```python
from build123d import *

# Parameters (mm, degrees)
SKETCH1_R           = 50
BOSS_EXTRUDE1_DEPTH = 5
SKETCH2_R           = 5
CUT_EXTRUDE1_DEPTH  = 5
CIRPATTERN1_COUNT   = 3
SKETCH3_R           = 9
CUT_EXTRUDE2_DEPTH  = 5


with BuildPart() as part:
    # Sketch1 → Boss-Extrude1 (new body)
    with BuildSketch(Plane.XY):
        Circle(SKETCH1_R)
    extrude(amount=BOSS_EXTRUDE1_DEPTH)

    # Sketch2 → Cut-Extrude1 (cut)
    with BuildSketch(Plane.XY.offset(5)):
        with Locations((0, 35)):
            Circle(SKETCH2_R)
    cut_extrude1 = extrude(amount=-CUT_EXTRUDE1_DEPTH, mode=Mode.SUBTRACT)

    # CirPattern1: Cut-Extrude1 ×3 about axis
    cirpattern1_axis = Axis((0, 0, 0), (0, 0, 1))
    for i in range(1, CIRPATTERN1_COUNT):
        add(cut_extrude1.rotate(cirpattern1_axis, i * 360 / CIRPATTERN1_COUNT), mode=Mode.SUBTRACT)

    # Sketch3 → Cut-Extrude2 (cut)
    with BuildSketch(Plane.XY.offset(5)):
        Circle(SKETCH3_R)
    extrude(amount=-CUT_EXTRUDE2_DEPTH, mode=Mode.SUBTRACT)


solid = part.part
```
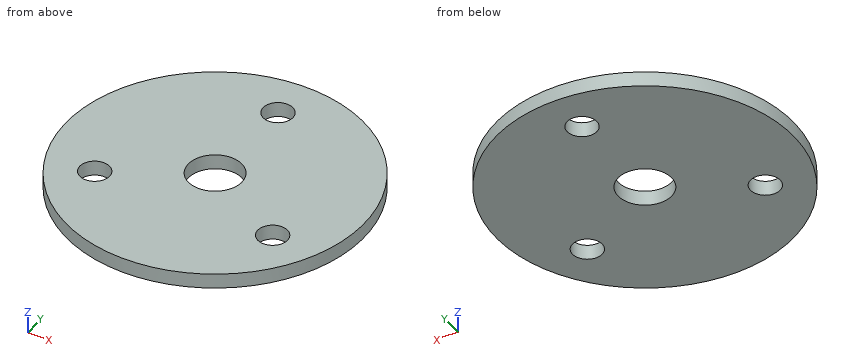
Input: part model. Units: mm. Frame: model coordinates. Give positions to 0.01 mm unless a question says otherwise; leave off trailing zeros. Order: outer loops, then holes, each group sorted by start corner. A loop starts at its lowest first (then second) coordinate and runs counter-clockwise, first axis right, second up.
1. Cut plane A-A (y = 0). Return loops of the section in (x, z).
Computed:
outline: (-50, 0) - (-9, 0) - (-9, 5) - (-50, 5) - close; (9, 0) - (50, 0) - (50, 5) - (9, 5) - close
2. Cut plane B-B (x = 0). Return loops of the section in (y, z), and give its area (3 significant figures).
Computed:
outline: (-50, 0) - (-9, 0) - (-9, 5) - (-50, 5) - close; (9, 0) - (30, 0) - (30, 5) - (9, 5) - close; (40, 0) - (50, 0) - (50, 5) - (40, 5) - close
area: 360 mm2
3. Line query: probe 1 along Y at (x, z) = (0, 3.25); probe 2 along X at (y, z) = (-0.5, 1.55); probe 3 along Y at (x, z) = (3, 0.4). Output: solid intervals per line, ascending.
Computed:
probe 1: y = -50 to -9, 9 to 30, 40 to 50
probe 2: x = -50 to -8.99, 8.99 to 50
probe 3: y = -49.91 to -8.49, 8.49 to 31, 39 to 49.91
4. Cut plane D-D (y = 35). Return loops of the section in (x, z), and give its area (3 significant figures).
Computed:
outline: (-35.71, 0) - (-5, 0) - (-5, 5) - (-35.71, 5) - close; (5, 0) - (35.71, 0) - (35.71, 5) - (5, 5) - close
area: 307 mm2
5. Pin query (flat end, axial travel): pin 1 Ø3 at (x, z) = (-17.5, 3) entering from -Y. Return the tip coordinate at first contact, or that it passes through.
Computed:
pin 1: stops at y = -47.37
6. Cut plane C-C (y = -20.5). Return loops of the section in (x, z).
Computed:
outline: (-45.6, 0) - (-34.31, 0) - (-34.31, 5) - (-45.6, 5) - close; (-26.31, 0) - (26.31, 0) - (26.31, 5) - (-26.31, 5) - close; (34.31, 0) - (45.6, 0) - (45.6, 5) - (34.31, 5) - close
